Answer from the drawing. Dimensions are ordinates in mm from the lowest x, y and z of the part. Round coordinates to 2 decimals unless told otherwise and drop trailing zeros. Write each loop counter-clockwise with the first axis right and the second up, starting at its lowest first coordinate (ties: lowest second). Pieces come first, ordered by that corner, then holes. Notation, with made-up numbers: (35, -20.5) - (81, -20.5) arc R5 cw to (81, -13.5) - close; hole circle Ø5 at (77.5, -5.75). An arc over 180 degrees is marked (long way). Use a Markdown table: item, result. Add a question column.
1) A cutting plane is placed at D-D (x = 10). Give the vertices of the cut face in (y, z), then the cut area to 3 significant figures.
2) A cutting plane is placed at A-A (y = 70). Give the vertices of the cut face in (x, z).
3) A cutting plane is placed at C-C (z = 3.5). Give the vertices of the cut face in (x, y).
4) Find the intervals of material crossed by probe 1 along X at (y, z) = (10, 7); probe 2 along Y at (x, z) = (70, 2.5), in increasing order. Write a range as from..to.
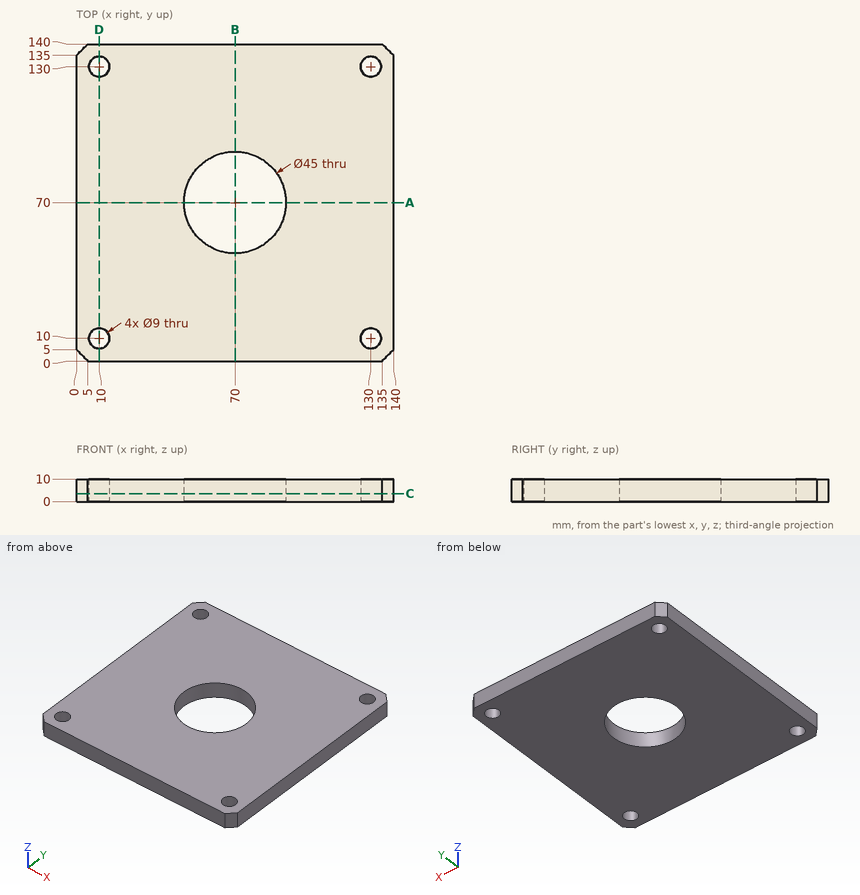
Entries:
| question | item | result |
|---|---|---|
| 1 | outline | (0, 0) - (5.5, 0) - (5.5, 10) - (0, 10) - close; (14.5, 0) - (125.5, 0) - (125.5, 10) - (14.5, 10) - close; (134.5, 0) - (140, 0) - (140, 10) - (134.5, 10) - close |
| 1 | area | 1,220 mm² |
| 2 | outline | (0, 0) - (47.5, 0) - (47.5, 10) - (0, 10) - close; (92.5, 0) - (140, 0) - (140, 10) - (92.5, 10) - close |
| 3 | outline | (0, 5) - (5, 0) - (135, 0) - (140, 5) - (140, 135) - (135, 140) - (5, 140) - (0, 135) - close; hole circle Ø9 at (10, 10); hole circle Ø9 at (10, 130); hole circle Ø45 at (70, 70); hole circle Ø9 at (130, 10); hole circle Ø9 at (130, 130) |
| 4 | probe 1 | x = 0..5.5, 14.5..125.5, 134.5..140 |
| 4 | probe 2 | y = 0..47.5, 92.5..140 |
